Can you work these out from the model? Positions are in its coordinate system, mm. A direction names the side the tool comes from. Give positions to 0.01 mm unless a question says otherwise; leave off trailing zeros. Loops run counter-clockwise (first coordinate to the right, second up) from the corner with the lowest first, then second, coordinate; pieces in that order, holes last. Notation, with made-up numbers: (-33.75, 65) - (-6.75, 65) arc R24 ccw to (-6.75, 90) - close; hole circle Ø4 at (84.25, 28). An arc over 180 degrees is marked (long way). Answer in a Markdown table with one row per item.
from build123d import *

# Parameters (mm, degrees)
CUT_EXTRUDE_1_DEPTH = 4


with BuildPart() as part:
    # 草图1 → 旋转1 (revolve)
    with BuildSketch(Plane.XY, mode=Mode.PRIVATE) as revolve_1_sk:
        with BuildLine():
            Line((0, 0), (0, 19))
            Line((0, 19), (1, 20))
            Line((1, 20), (3.05, 20))
            Line((3.05, 20), (3.05, 19))
            Line((3.05, 19), (5, 19))
            Line((5, 19), (5, 20))
            Line((5, 20), (22.75, 20))
            ThreePointArc((22.75, 20), (22.926776695, 20.073223305), (23, 20.25))
            Line((23, 20.25), (23, 24))
            Line((23, 24), (24, 25))
            Line((24, 25), (1137, 25))
            Line((1137, 25), (1138, 24))
            Line((1138, 24), (1138, 20))
            Line((1138, 20), (1230, 20))
            Line((1230, 20), (1231, 19))
            Line((1231, 19), (1231, 15))
            Line((1231, 15), (1280, 15))
            Line((1280, 15), (1281, 14))
            Line((1281, 14), (1281, 0))
            Line((1281, 0), (0, 0))
        make_face()
    revolve(revolve_1_sk.sketch.rotate(Axis((1281, 0, 0), (-1, 0, 0)), 270), axis=Axis((1281, 0, 0), (-1, 0, 0)))

    # 草图2 → 切除-拉伸1 (cut)
    with BuildSketch(Plane(origin=(0, 15, 0), x_dir=(1, 0, 0), z_dir=(0, 1, 0))):
        with BuildLine():
            Line((1240, -4), (1272, -4))
            ThreePointArc((1272, -4), (1276, 0), (1272, 4))
            Line((1272, 4), (1240, 4))
            ThreePointArc((1240, 4), (1236, 0), (1240, -4))
        make_face()
    extrude(amount=-CUT_EXTRUDE_1_DEPTH, mode=Mode.SUBTRACT)


solid = part.part
Q1. If I drill on line 1 (Z direction, x = 1205, y = -5.5); line 2 (X direction, y = 16.5, z = -3); line 3 (X direction, y = 10, z = 11), over which ranges is the centre line in solid material (lowest first)? Write a range as [from, to].
Checked values:
| item | result |
|---|---|
| line 1 | z = [-19.23, 19.23] |
| line 2 | x = [0, 1231] |
| line 3 | x = [0, 1280.13] |
Q2. On a 3-axis mill with a long thin cutter (end or side, diameter ignored), from which of +Z, -Z, +X, -X, +Y, -Y can I reach the whole of each face in a straight line? I mean faces 1 (the face through (13.999, -19.524, -4.336)), 2 (the face through (4.04, -11.56, -15.08)), 3 (the face through (1231, 6, 14)). Say none if no direction works.
Checked values:
| item | result |
|---|---|
| face 1 | -X |
| face 2 | none |
| face 3 | +X |
Q3. For pin 1 (8 mm diameter, centred on x = 1091.5, y = 13, fed in from -Z); pin 2 (6 mm diameter, centred on y = 13.5, z = -14.5, fed in from +X); pin 3 (3 mm diameter, centred on x = 1151, y = -18.5, fed in from -Z), each with a flat end and sliding along its axis, tell me the tip position at first contact or that it passes through.
Checked values:
| item | result |
|---|---|
| pin 1 | stops at z = -23.32 |
| pin 2 | stops at x = 1231 |
| pin 3 | stops at z = -10.54 |
Q4. Imagine slicing it at A-A, the plane x = 1103. Write out the boundary of the cut face in (y, z).
Checked values:
| item | result |
|---|---|
| outline | circle Ø50 at (0, 0) |
